from build123d import *

# Parameters (mm, degrees)
BRACKET_BODY_DEPTH     = 31
HEAD_CHAMFER_SKETCH_R  = 3.5
HEAD_CHAMFER_CUT_DEPTH = 31
HEAD_NOTCH_SKETCH_W    = 7
HEAD_NOTCH_SKETCH_H    = 11
HEAD_NOTCH_CUT_DEPTH   = 51
FORKED_SLOT_CUT_DEPTH  = 102


with BuildPart() as part:
    # Bracket Profile Sketch → Bracket Body (new, symmetric)
    with BuildSketch(Plane.XY):
        Polygon((0, 15), (0, 0), (27, 0), (112, 0), (112, 15), (27, 15), (27, 42), (0, 42), align=None)
    extrude(amount=BRACKET_BODY_DEPTH, both=True)

    # Head Chamfer Sketch → Head Chamfer Cut (cut, symmetric)
    with BuildSketch(Plane(origin=(27, 0, 0), x_dir=(0, 0, -1), z_dir=(1, 0, 0))):
        with Locations(Location((0, 33, 0), (0, 0, 180))):
            Circle(HEAD_CHAMFER_SKETCH_R)
        Polygon((10.202979839, 42), (31, 30.94202823), (31, 54.961145536), (-31, 54.961145536), (-31, 30.940443821), (-10.2, 42), align=None)
    extrude(amount=HEAD_CHAMFER_CUT_DEPTH, both=True, mode=Mode.SUBTRACT)

    # Head Notch Sketch → Head Notch Cut (cut, symmetric)
    with BuildSketch(Plane(origin=(0, 42, 0), x_dir=(1, 0, 0), z_dir=(0, 1, 0))):
        with Locations((3.5, 25.5)):
            Rectangle(HEAD_NOTCH_SKETCH_W, HEAD_NOTCH_SKETCH_H)
        with Locations((3.5, -25.5)):
            Rectangle(HEAD_NOTCH_SKETCH_W, HEAD_NOTCH_SKETCH_H)
    extrude(amount=HEAD_NOTCH_CUT_DEPTH, both=True, mode=Mode.SUBTRACT)

    # Forked Slot Sketch → Forked Slot Cut (cut)
    with BuildSketch(Plane(origin=(0, 15, 0), x_dir=(1, 0, 0), z_dir=(0, 1, 0))):
        Polygon((62, -31), (112, -23), (112, -31), align=None)
        Polygon((62, 31), (112, 23), (112, 31), align=None)
        with BuildLine():
            Line((83, 9), (112, 9))
            Line((112, 9), (112, -9))
            Line((112, -9), (83, -9))
            ThreePointArc((83, -9), (74, 0), (83, 9))
        make_face()
    extrude(amount=-FORKED_SLOT_CUT_DEPTH, mode=Mode.SUBTRACT)


solid = part.part
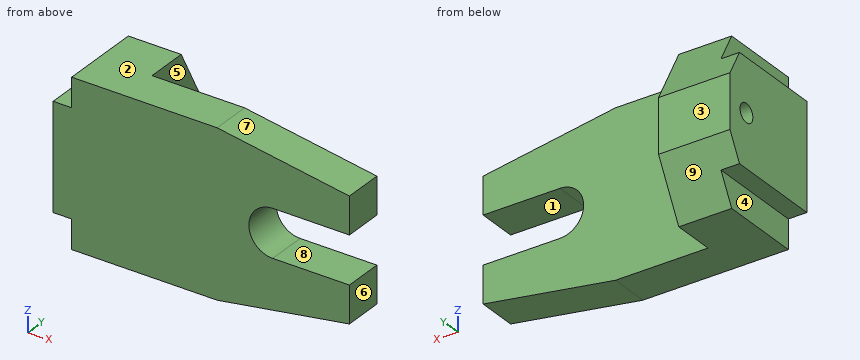
The model under review builds one solid part; all positions refer to its coordinate system, in mm. Face numbers are marked on the shaded views. A direction names the side the tool comes from. Round coordinates to 2 decimals unless told otherwise and drop trailing zeros. Order: outer loops, then holes, each group sorted by start corner. A loop starts at its lowest first (then second) coordinate and runs counter-clockwise, first axis right, second up. Notation, with made-up numbers: (40.25, -14) -> (97.25, -14) arc R9 cw to (97.25, 0) -> close; hole circle Ø8 at (-32.75, 88). An arc over 180 degrees is marked (long way). Use CSV: the item, a comma, the result in double quotes. Start each with the question number.
(1) Consider section D-D on x = 101. Write out the cut boundary in (y, z).
(2) Consider section B-B on z = 0. Write out the cut boundary in (x, y), and give its area (3 significant figures).
(3) Consider section C-C on y = 8.5. Write out the cut boundary in (x, z).
(4) Insertion check: pin 1 (12 mm diameter, centred on x = 91.5, y = 11, fed in from -Z); pin 2 (2 mm diameter, centred on x = 5, y = 9, fed in from -Z); pin 3 (1 mm diameter, centred on x = 64.5, y = 16, fed in from -Z); pin 4 (16.5 mm diameter, centred on x = 99.5, y = 6.5, fed in from +Z). Each pin has a flat end and moves straight along its axis. Give the tip position at first contact, or say it passes through.
(5) Mouldability with a two-part tool opening along Z and no side actions: class the marked faces 6, 7, 8 and 9 as pulls with the +Z half, pulls with the -Z half, needs draft (parallel to the pull), parting line crosses it, or undercut.
(6) Consider section A-A on x = 86. Write out the cut boundary in (y, z).
(7) Wall thickness on probe 1 along Y at (x, z) = (13.5, 0); probe 2 along Y at (x, z) = (96, 23.5); probe 3 along X at (y, z) = (19.5, 16): over which ranges is each line inside the solid? List them lowest first. Write a range as from..to.
(8) Tool access review of the marked faces 1, 2, 3, 4 and 5: name each direction out of +Z, -Z, +X, -X, +Y, -Y from which nothing blocks a thin tool from reaching the whole face with its end or side.
Responses:
1,outline,"(0, -24.76) -> (15, -24.76) -> (15, -9) -> (0, -9) -> close; (0, 9) -> (15, 9) -> (15, 24.76) -> (0, 24.76) -> close"
2,outline,"(0, 0) -> (74, 0) -> (74, 15) -> (27, 15) -> (27, 29.5) -> (0, 29.5) -> close; (0, 36.5) -> (27, 36.5) -> (27, 42) -> (0, 42) -> close"
2,area,"1,650 mm²"
3,outline,"(0, -20) -> (7, -20) -> (7, -31) -> (62, -31) -> (112, -23) -> (112, -9) -> (83, -9) arc R9 cw to (83, 9) -> (112, 9) -> (112, 23) -> (62, 31) -> (7, 31) -> (7, 20) -> (0, 20) -> close"
4,pin 1,"z = -27.24"
4,pin 2,"z = -20"
4,pin 3,"through"
4,pin 4,"z = 26.32"
5,face 6,"needs draft"
5,face 7,"pulls with the +Z half"
5,face 8,"undercut"
5,face 9,"pulls with the -Z half"
6,outline,"(0, -27.16) -> (15, -27.16) -> (15, -9) -> (0, -9) -> close; (0, 9) -> (15, 9) -> (15, 27.16) -> (0, 27.16) -> close"
7,probe 1,"0..29.5, 36.5..42"
7,probe 2,"0..15"
7,probe 3,"0..27"
8,face 1,"+X, +Y, -Y"
8,face 2,"+Z, +X, -X, +Y, -Y"
8,face 3,"+Z, -Z, +X, -X, +Y"
8,face 4,"-Z, -X, +Y, -Y"
8,face 5,"+Z, -Z, +X, +Y"
